```python
from build123d import *

# Parameters (mm, degrees)
SKETCH_1_R              = 20
EXTRUDE_1_DEPTH         = 2286
HOLE_WIZARD_M14_1_D     = 12
HOLE_WIZARD_M14_1_DEPTH = 34
HOLE_WIZARD_M14_1_TIP   = 3.605163714
HOLE_WIZARD_M14_2_D     = 12
HOLE_WIZARD_M14_2_DEPTH = 34
HOLE_WIZARD_M14_2_TIP   = 3.605163714


with BuildPart() as part:
    # 草图1 → 凸台-拉伸1 (new body)
    with BuildSketch(Plane(origin=(0, 0, 0), x_dir=(1, 0, 0), z_dir=(0, 1, 0))):
        with Locations(Location((0, 0, 0), (0, 0, 270))):
            Circle(SKETCH_1_R)
    extrude(amount=EXTRUDE_1_DEPTH)

    # M14 螺纹孔1
    with Locations(Plane(origin=(0, 2286, 0), x_dir=(1, 0, 0), z_dir=(0, 1, 0))):
        with Locations((0, 0)):
            Hole(HOLE_WIZARD_M14_1_D / 2, depth=HOLE_WIZARD_M14_1_DEPTH)
            with Locations((0, 0, -(HOLE_WIZARD_M14_1_DEPTH + HOLE_WIZARD_M14_1_TIP / 2))):  # 118° drill point
                Cone(0, HOLE_WIZARD_M14_1_D / 2, HOLE_WIZARD_M14_1_TIP, mode=Mode.SUBTRACT)

    # M14 螺纹孔2
    with Locations(Plane(origin=(0, 0, 0), x_dir=(-1, 0, 0), z_dir=(0, -1, 0))):
        with Locations((0, 0)):
            Hole(HOLE_WIZARD_M14_2_D / 2, depth=HOLE_WIZARD_M14_2_DEPTH)
            with Locations((0, 0, -(HOLE_WIZARD_M14_2_DEPTH + HOLE_WIZARD_M14_2_TIP / 2))):  # 118° drill point
                Cone(0, HOLE_WIZARD_M14_2_D / 2, HOLE_WIZARD_M14_2_TIP, mode=Mode.SUBTRACT)


solid = part.part
```
Input: part model. Units: mm. Frame: model coordinates. Give positions to 0.01 mm unless a question says otherwise; leave off trailing zeros. Order: outer loops, then holes, each group sorted by start corner. A loop starts at its lowest first (then second) coordinate and runs counter-clockwise, first axis right, second up. Notation, with made-up numbers: (67.25, 22.5) - (113.25, 22.5) arc R34 ccw to (113.25, 52.5) - close; hole circle Ø4 at (87, 69). An arc over 180 degrees is marked (long way). Use a Markdown table: item, result.
(1) Section query B-B (z = -13.5). Output: boundary loops of the cut face in (x, y).
Computed values:
| item | result |
|---|---|
| outline | (-14.76, 0) - (14.76, 0) - (14.76, 2286) - (-14.76, 2286) - close |
(2) Pin query (flat end, axial travel): pin 1 (8 mm diameter, centred on x = -6.5, y = 507, fed in from +Z); pin 2 (8 mm diameter, centred on x = 6, y = 1079, fed in from +Z); pin 3 (9.5 mm diameter, centred on x = 0, z = 0, fed in from -Y). Return the tip coordinate at first contact, or that it passes through.
Computed values:
| item | result |
|---|---|
| pin 1 | stops at z = 19.84 |
| pin 2 | stops at z = 19.9 |
| pin 3 | stops at y = 34.75 |
(3) Section query A-A (y = 980). Output: boundary loops of the cut face in (x, z).
Computed values:
| item | result |
|---|---|
| outline | circle Ø40 at (0, 0) |
(4) Line query: line 1 (Z direction, x = 2, y = 1806.5); line 2 (X direction, y = 2155, z = -1); line 3 (X direction, y = 660, z = -8). Output: solid intervals per line, ascending. Write a range as from..to.
Computed values:
| item | result |
|---|---|
| line 1 | z = -19.9..19.9 |
| line 2 | x = -19.97..19.97 |
| line 3 | x = -18.33..18.33 |
